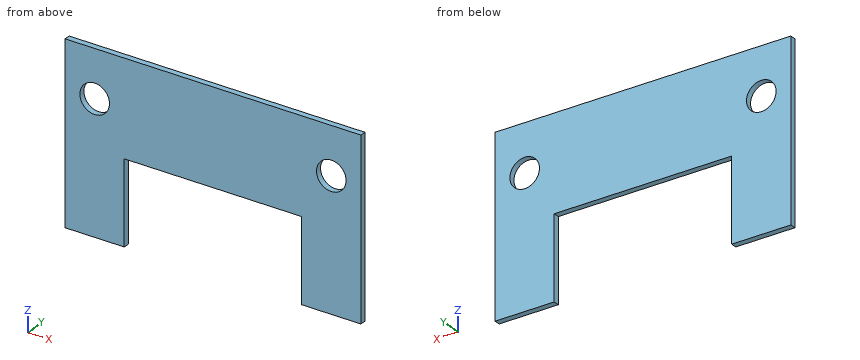
```python
from build123d import *

# Parameters (mm, degrees)
SKETCH1_R           = 1.25
BOSS_EXTRUDE1_DEPTH = 0.5


with BuildPart() as part:
    # Sketch1 → Boss-Extrude1 (new body)
    with BuildSketch(Plane(origin=(0, 0, 0), x_dir=(1, 0, 0), z_dir=(0, 1, 0))):
        Polygon((-12.5, 0), (12.5, 0), (12.5, 15), (7.5, 15), (7.5, 8), (-7.5, 8), (-7.5, 15), (-12.5, 15), align=None)
        with Locations(Location((10, 4, 0), (0, 0, 270))):
            Circle(SKETCH1_R, mode=Mode.SUBTRACT)
        with Locations(Location((-10, 4, 0), (0, 0, 270))):
            Circle(SKETCH1_R, mode=Mode.SUBTRACT)
    extrude(amount=BOSS_EXTRUDE1_DEPTH)


solid = part.part
```
Verification items for the finished model (mm, model axes). Give positions to 0.01 mm unless a question says otherwise; leave off trailing zeros. Write each loop counter-clockwise with the first axis right and the second up, starting at its lowest first coordinate (ties: lowest second). Pieces come first, ordered by that corner, then holes. Notation, with made-up numbers: M -38,-15.75 L -21,-15.75 A21 ccw -21,-8.75 Z; hole C 41,48 d2. An arc over 180 degrees is marked long. One line per question, with ' | ' between items.
1) Section check B-B on x = 10. Enter the section's corners in (y, z), plus the area to 3 significant figures.
Result:
outline: M 0,-15 L 0.5,-15 L 0.5,-5.25 L 0,-5.25 Z; M 0,-2.75 L 0.5,-2.75 L 0.5,0 L 0,0 Z | area: 6.25 mm2
2) Thickness scan on line 1 along X through (y, z) = (0.2, -4); line 2 along X through (y, z) = (0.2, -14.25); line 3 along X through (y, z) = (0.1, -3.5). Record the ranges inside material, lowest first. Write a range as [from, to].
Result:
line 1: x = [-12.5, -11.25], [-8.75, 8.75], [11.25, 12.5] | line 2: x = [-12.5, -7.5], [7.5, 12.5] | line 3: x = [-12.5, -11.15], [-8.85, 8.85], [11.15, 12.5]
3) Section check A-A on z = -3. Enter the section's corners in (x, y), plus the area to 3 significant figures.
Result:
outline: M -12.5,0 L -10.75,0 L -10.75,0.5 L -12.5,0.5 Z; M -9.25,0 L 9.25,0 L 9.25,0.5 L -9.25,0.5 Z; M 10.75,0 L 12.5,0 L 12.5,0.5 L 10.75,0.5 Z | area: 11.0 mm2
4) Section check D-D on x = -9.5. Enter the section's corners in (y, z), plus the area to 3 significant figures.
Result:
outline: M 0,-15 L 0.5,-15 L 0.5,-5.15 L 0,-5.15 Z; M 0,-2.85 L 0.5,-2.85 L 0.5,0 L 0,0 Z | area: 6.35 mm2
5) Gauge pin test, flat end, axial feed: pin 1 Ø1 at (x, z) = (5.5, -11.5) entering from +Y. Record the tip position at first contact, or that the pin passes through.
Result:
pin 1: passes through
6) Section check C-C on y = 0.1. Enter the section's corners in (x, z), plus the area to 3 significant figures.
Result:
outline: M -12.5,-15 L -7.5,-15 L -7.5,-8 L 7.5,-8 L 7.5,-15 L 12.5,-15 L 12.5,0 L -12.5,0 Z; hole C -10,-4 d2.5; hole C 10,-4 d2.5 | area: 260 mm2
